from build123d import *

# Parameters (mm, degrees)
SKETCH_1_W                   = 140
SKETCH_1_H                   = 40
EXTRUDE_1_DEPTH              = 16
HOLE_WIZARD_M10_1_D          = 8.5
HOLE_WIZARD_M8_1_D           = 8.4
HOLE_WIZARD_M8_1_CBORE_D     = 15
HOLE_WIZARD_M8_1_CBORE_DEPTH = 8.6
CHAMFER_1_SIZE               = 2


with BuildPart() as part:
    # 草图1 → 凸台-拉伸1 (new body)
    with BuildSketch(Plane.XY):
        with Locations((70, 20)):
            Rectangle(SKETCH_1_W, SKETCH_1_H)
    extrude(amount=EXTRUDE_1_DEPTH)

    # M10 螺纹孔1 (through all)
    with Locations(Plane(origin=(0, 40, 0), x_dir=(1, 0, 0), z_dir=(0, 1, 0))):
        with Locations((40, -8), (100, -8)):
            Hole(HOLE_WIZARD_M10_1_D / 2)

    # M8 六角凹头螺钉的柱形沉头孔1 (through all)
    with Locations(Plane.XY.offset(16)):
        with Locations((20, 10), (120, 10)):
            CounterBoreHole(HOLE_WIZARD_M8_1_D / 2, HOLE_WIZARD_M8_1_CBORE_D / 2, HOLE_WIZARD_M8_1_CBORE_DEPTH)

    # 倒角1
    chamfer_1_edges = [part.edges().sort_by_distance(p)[0] for p in [
        (140, 20, 16),
        (0, 20, 16),
        (140, 20, 0),
        (0, 20, 0),
    ]]
    chamfer(chamfer_1_edges, length=CHAMFER_1_SIZE)


solid = part.part
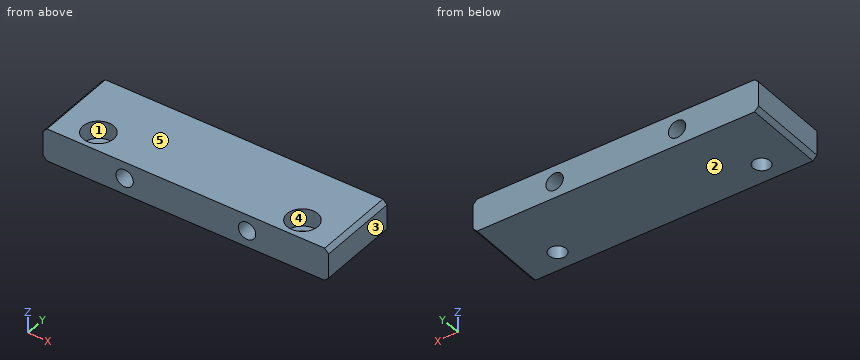
Can you work these out from the model? Positions are in its coordinate system, mm. Face numbers are marked on the shaded views. A direction names the side the tool comes from. Give positions to 0.01 mm unless a question says otherwise; leave off trailing zeros. Loops run counter-clockwise (first coordinate to the right, second up) from the corner with the lowest first, then second, coordinate; pieces in that order, holes last. Notation, with made-up numbers: (17.25, 41.25) -> (41.25, 41.25) arc R29 ccw to (41.25, 76.25) -> close; hole circle Ø2 at (-1.5, -12). An arc over 180 degrees is marked (long way). Return JSON: item names as keys, results as strings.
Q1. I want a section at D-D, the plane y = 27.5. List the corners of the cut face in (x, z) for me, then the cut area to 3 significant figures.
Checks:
{"outline": "(0, 2) -> (2, 0) -> (138, 0) -> (140, 2) -> (140, 14) -> (138, 16) -> (2, 16) -> (0, 14) -> close; hole circle Ø8.5 at (40, 8); hole circle Ø8.5 at (100, 8)", "area": "2,120 mm2"}
Q2. For pin 1 Ø7.5 at (x, z) = (100, 8) entering from -Y; pin 2 Ø12 at (x, y) = (20, 10) entering from +Z, each with a flat end and sliding along its axis, tell me the tip position at first contact or that it passes through.
Checks:
{"pin 1": "passes through", "pin 2": "stops at z = 7.4"}
Q3. We'd pull the mould along X, two halves only. Please class the marked faces 3, 4 and 5: released by +X, released by -X, zero draft, split by the parting line, or undercut.
Checks:
{"face 3": "released by +X", "face 4": "undercut", "face 5": "zero draft"}
Q4. I want a section at C-C, the plane x = 40. List the corners of the cut face in (y, z) for me.
Checks:
{"outline": "(0, 0) -> (40, 0) -> (40, 3.75) -> (0, 3.75) -> close; (0, 12.25) -> (40, 12.25) -> (40, 16) -> (0, 16) -> close"}
Q5. I need wall thicknesses on probe 1 along Y at (x, z) = (20, 4); probe 2 along X at (y, z) = (16.5, 8.5); probe 3 along X at (y, z) = (12, 5). Which ranges of each line are inside material? Lowest first, please.
Checks:
{"probe 1": "y = 0 to 5.8, 14.2 to 40", "probe 2": "x = 0 to 16.26, 23.74 to 35.78, 44.22 to 95.78, 104.22 to 116.26, 123.74 to 140", "probe 3": "x = 0 to 16.31, 23.69 to 36.99, 43.01 to 96.99, 103.01 to 116.31, 123.69 to 140"}
Q6. On a 3-axis mill with a long thin cutter (end or side, diameter ignored), from which of +Z, -Z, +X, -X, +Y, -Y can I reach the whole of each face in a straight line? I mean the marked faces 1 and 2. Say none if no direction works.
Checks:
{"face 1": "+Z", "face 2": "-Z, +X, -X, +Y, -Y"}
Q7. I want a section at A-A, the plane y = 10. List the corners of the cut face in (x, z) for me, then the cut area to 3 significant figures.
Checks:
{"outline": "(0, 2) -> (2, 0) -> (15.8, 0) -> (15.8, 7.4) -> (12.5, 7.4) -> (12.5, 16) -> (2, 16) -> (0, 14) -> close; (24.2, 0) -> (115.8, 0) -> (115.8, 7.4) -> (112.5, 7.4) -> (112.5, 16) -> (27.5, 16) -> (27.5, 7.4) -> (24.2, 7.4) -> close; (124.2, 0) -> (138, 0) -> (140, 2) -> (140, 14) -> (138, 16) -> (127.5, 16) -> (127.5, 7.4) -> (124.2, 7.4) -> close; hole circle Ø8.5 at (40, 8); hole circle Ø8.5 at (100, 8)", "area": "1,740 mm2"}
Q8. I want a section at B-B, the plane z = 10. List the corners of the cut face in (x, y) for me.
Checks:
{"outline": "(0, 0) -> (36.25, 0) -> (36.25, 40) -> (0, 40) -> close; (43.75, 0) -> (96.25, 0) -> (96.25, 40) -> (43.75, 40) -> close; (103.75, 0) -> (140, 0) -> (140, 40) -> (103.75, 40) -> close; hole circle Ø15 at (20, 10); hole circle Ø15 at (120, 10)"}
